from build123d import *

# Parameters (mm, degrees)
BASE_PLATE_DEPTH         = 15
UPPER_PLATE_DEPTH        = 10
LOOP_WALL_DEPTH          = 50
LOOP_WALL_DEPTH_BACK     = 10
WALL_OPENING_CUT_DEPTH   = 160
TAB_SKETCH_W             = 25
TAB_SKETCH_H             = 10
TAB_DEPTH                = 20
GUIDE_RAIL_1_DEPTH       = 7
GUIDE_RAIL_1_DEPTH_BACK  = 3
GUIDE_RAIL_2_DEPTH       = 7
GUIDE_RAIL_2_DEPTH_BACK  = 3
ANGLED_TRIM_CUT_SKETCH_R = 15
ANGLED_TRIM_CUT_DEPTH    = 133.5


with BuildPart() as part:
    # Base Plate Sketch → Base Plate (new body)
    with BuildSketch(Plane(origin=(0, 0, 0), x_dir=(1, 0, 0), z_dir=(0, 1, 0))):
        with BuildLine():
            Line((-50, 50), (50, 50))
            ThreePointArc((50, 50), (100, 0), (50, -50))
            Line((50, -50), (-50, -50))
            ThreePointArc((-50, -50), (-100, 0), (-50, 50))
        make_face()
    extrude(amount=BASE_PLATE_DEPTH)



with BuildPart() as body_2:
    # Upper Plate Sketch → Upper Plate (new body)
    with BuildSketch(Plane(origin=(0, 80, 0), x_dir=(1, 0, 0), z_dir=(0, 1, 0))):
        with BuildLine():
            Line((50, 50), (25, 50))
            Line((25, 50), (25, 25))
            Line((25, 25), (-50, 25))
            ThreePointArc((-50, 25), (-75, 0), (-50, -25))
            Line((-50, -25), (50, -25))
            ThreePointArc((50, -25), (75, 0), (50, 25))
            Line((50, 25), (50, 50))
        make_face()
    extrude(amount=UPPER_PLATE_DEPTH)

    # Loop Wall Sketch → Loop Wall (add, two sides: drawn at the far end of the back side and taken through both)
    with BuildSketch(Plane(origin=(0, 90, 0), x_dir=(1, 0, 0), z_dir=(0, 1, 0)).offset(-LOOP_WALL_DEPTH_BACK)):
        with BuildLine():
            Line((-50, 50), (50, 50))
            ThreePointArc((50, 50), (100, 0), (50, -50))
            Line((50, -50), (-50, -50))
            ThreePointArc((-50, -50), (-100, 0), (-50, 50))
        make_face()
        with BuildLine():
            Line((-50, 40), (50, 40))
            ThreePointArc((50, 40), (90, 0), (50, -40))
            Line((50, -40), (-50, -40))
            ThreePointArc((-50, -40), (-90, 0), (-50, 40))
        make_face(mode=Mode.SUBTRACT)
    extrude(amount=LOOP_WALL_DEPTH + LOOP_WALL_DEPTH_BACK)

    # Wall Opening Cut Sketch → Wall Opening Cut (cut, symmetric)
    with BuildSketch(Plane.XY.offset(50)):
        Polygon((100, 90), (-100, 125.265396142), (-100, 140), (100, 140), align=None)
    extrude(amount=WALL_OPENING_CUT_DEPTH, both=True, mode=Mode.SUBTRACT)

    # Tab Sketch → Tab (add)
    with BuildSketch(Plane.XY.offset(25)):
        with Locations((-37.5, 85)):
            Rectangle(TAB_SKETCH_W, TAB_SKETCH_H)
    extrude(amount=TAB_DEPTH)


with BuildPart() as part_1:
    add(part.part)

    add(body_2.part)  # Guide Rail 1 merges body 2
    # Guide Rail 1 Sketch → Guide Rail 1 (add, two sides: drawn at the far end of the back side and taken through both)
    with BuildSketch(Plane.XY.offset(-40).offset(-GUIDE_RAIL_1_DEPTH_BACK)):
        Polygon((50, 15), (75, 15), (-50, 80), (-75, 80), align=None)
    extrude(amount=GUIDE_RAIL_1_DEPTH + GUIDE_RAIL_1_DEPTH_BACK)

    # Guide Rail 2 Sketch → Guide Rail 2 (add, two sides: drawn at the far end of the back side and taken through both)
    with BuildSketch(Plane(origin=(0, 0, 40), x_dir=(-1, 0, 0), z_dir=(0, 0, -1)).offset(-GUIDE_RAIL_2_DEPTH_BACK)):
        Polygon((50, 15), (75, 15), (-50, 80), (-75, 80), align=None)
    extrude(amount=GUIDE_RAIL_2_DEPTH + GUIDE_RAIL_2_DEPTH_BACK)

    # Angled Trim Cut Sketch → Angled Trim Cut (cut, symmetric)
    with BuildSketch(Plane(origin=(0, 15, 0), x_dir=(1, 0, 0), z_dir=(0, 1, 0))):
        with Locations(Location((-50, 0, 0), (0, 0, 270))):
            Circle(ANGLED_TRIM_CUT_SKETCH_R)
        with Locations(Location((50, 0, 0), (0, 0, 270))):
            Circle(ANGLED_TRIM_CUT_SKETCH_R)
    extrude(amount=ANGLED_TRIM_CUT_DEPTH, both=True, mode=Mode.SUBTRACT)


solid = part_1.part
Source: CAD feature listing. Evaluate the final solid. Frame: model axes, mm. A direction names the side the tool comes from. Coordinates: 2 decimals unless noted, no trailing zeros. Loops run counter-clockwise (first coordinate to the right, second up) from the corner with the lowest first, then second, coordinate; pieces in that order, holes last. Notation, with made-up numbers: (-22, 48) - (29, 48) arc R8 ccw to (29, 52) - close; hole circle Ø8 at (76.5, 25.5). An arc over 180 degrees is marked (long way). One line per item, written item: value. Start each with the question number.
1. Section C-C (z = -4.5). State how many separate pieces and enclosed holes the cut face has, and give its area (3 significant figures).
2. Mould query, pull axis Z, two halves, no side actions, for faces 4 (the flat face through (50, 85, -32)), 5 (the flat face through (-1, 7, -50)), 6 (the flat face through (1, 94, 50)). Classes: pulls with the +Z half, pulls with the -Z half, needs draft (parallel to the pull), parting line crosses it, or undercut.
3. Ray query, L1, parallel to X at y = 83, z = 0; L2, parallel to X at y = 6.75, z = 0; L3, parallel to Y at x = -73.5, z = 2.5. Return the intervals inside material, ascending.
4. Contact query for flat-ended pins moving along their axis: P1, Ø8, axis at y = 86, z = 35.5, coming from the +X side; P2, Ø3, axis at y = 103.5, z = 36.5, coming from the -X side; P3, Ø3, axis at y = 85, z = 35.5, coming from the -X side. Output: stop coordinate, or through.
5. Set-up query: faces 1 (the flat face through (0, 48, -43)), 2 (the cylindrical face through (-37.35, 7.6, 8.06)), 3 (the flat face through (59, 80, 36)). Return all of +Z, -Z, +X, -X, +Y, -Y with unobstructed straight access to the full face (end or side cutting, diameter ignored); none if empty.
6. Section A-A (x = 19.5). Return the cut outline in (y, z).
7. Section B-B (y = 44). Return the cut outline in (x, z), and give its area (3 significant figures).
Verdict:
1. separate pieces: 8
1. enclosed holes: 0
1. area: 3,610 mm2
2. face 4: undercut
2. face 5: pulls with the -Z half
2. face 6: pulls with the +Z half
3. L1: x = -100 to -90, -75 to -65, -35 to 35, 65 to 75, 90 to 100
3. L2: x = -100 to -65, -35 to 35, 65 to 100
3. L3: y = 0 to 15, 80 to 90
4. P1: stops at x = 88.83
4. P2: stops at x = -85.71
4. P3: stops at x = -86.66
5. face 1: -Z, +X, -X
5. face 2: +Y, -Y
5. face 3: +Y
6. outline: (0, -50) - (15, -50) - (15, 50) - (0, 50) - close; (30.86, -43) - (43.86, -43) - (43.86, -33) - (30.86, -33) - close; (51.14, 33) - (64.14, 33) - (64.14, 43) - (51.14, 43) - close; (80, -50) - (104.19, -50) - (104.19, -40) - (80, -40) - close; (80, -25) - (90, -25) - (90, 25) - (80, 25) - close; (80, 40) - (104.19, 40) - (104.19, 50) - (80, 50) - close
7. outline: (-19.23, 33) - (5.77, 33) - (5.77, 43) - (-19.23, 43) - close; (-5.77, -43) - (19.23, -43) - (19.23, -33) - (-5.77, -33) - close
7. area: 500 mm2
